```python
from build123d import *


with BuildPart() as part:
    # Sketch1 → Revolve1 (revolve)
    with BuildSketch(Plane.XY, mode=Mode.PRIVATE) as revolve1_sk:
        with BuildLine():
            Line((-4.9, 0), (-4.80754717, 3.5))
            Line((-4.80754717, 3.5), (-4.6, 3.5))
            Line((-4.6, 3.5), (-4.6, 4))
            Line((-4.6, 4), (-4.794339623, 4))
            Line((-4.794339623, 4), (-4.203177883, 26.379694424))
            ThreePointArc((-4.203177883, 26.379694424), (-4.171478034, 26.482572984), (-4.09103814, 26.554115293))
            ThreePointArc((-4.09103814, 26.554115293), (-2.09948154, 27.260450279), (0, 27.5))
            Line((0, 27.5), (0, 26.379694424))
            Line((0, 26.379694424), (-3.25, 26.379694424))
            Line((-3.25, 26.379694424), (-3.75, 1))
            Line((-3.75, 1), (-4, 1))
            Line((-4, 1), (-4, 0))
            Line((-4, 0), (-4.9, 0))
        make_face()
    revolve(revolve1_sk.sketch.rotate(Axis((0, 0, 0), (0, 1, 0)), 270), axis=Axis((0, 0, 0), (0, 1, 0)))


solid = part.part
```
Here's how the part is built. I have some questions about the finished solid (model axes, mm). A direction names the side the tool comes from. Round coordinates to 2 decimals unless told otherwise and drop trailing zeros. Loops run counter-clockwise (first coordinate to the right, second up) from the corner with the lowest first, then second, coordinate; pieces in that order, holes last. Notation, with made-up numbers: (4, 16) -> (22, 16) arc R19 cw to (22, 22) -> close; hole circle Ø5 at (43, 39.25). An arc over 180 degrees is marked (long way). Answer as CSV lines item,"result".
1. If we section it at B-B on y = 2.5: Please give me the cut outline in (x, z).
Final values:
outline,"circle Ø9.67 at (0, 0); hole circle Ø7.44 at (0, 0)"
2. Which directions (+Z, -Z, +X, -X, +Y, -Y) give clear straight access to the entire face, cutting with the end or side of a thin tool? Please do faces 1 (the face through (3.905, 0.493, 0.867)), 2 (the face through (4.74, 1.77, 1.05)).
Final values:
face 1,"-Y"
face 2,"+Y"
3. Thinking about a two-plate mould opening in Z: for faces 3 (the face through (-1.38, 3.75, -4.39)), 4 (the face through (4, 0, -2)), 5 (the face through (2.13, 13.51, 2.78)), 6 (the face through (0, 26.38, 0)), which applies, released by +Z, released by -Z, zero draft, split by the parting line, or undercut?
Final values:
face 3,"split by the parting line"
face 4,"zero draft"
face 5,"undercut"
face 6,"undercut"
4. If we section it at A-A on y = 14: Please give me the cut outline in (x, z), plus the area to 3 significant figures.
Final values:
outline,"circle Ø9.06 at (0, 0); hole circle Ø6.99 at (0, 0)"
area,"26.1 mm^2"
5. If I drill on L1, parallel to Z at x = 2, y = 6.75; L2, parallel to Z at x = 2.25, y = 7.75; L3, parallel to X at y = 0.3, z = 0, over which ranges is the centre line in solid material (lowest first)?
Final values:
L1,"z = -4.28 to -3.04, 3.04 to 4.28"
L2,"z = -4.12 to -2.83, 2.83 to 4.12"
L3,"x = -4.89 to -4, 4 to 4.89"
6. For pin 1 (5 mm diameter, centred on x = -1, y = 5.5, fed in from -Z); pin 2 (2 mm diameter, centred on x = -2, z = -1, fed in from +Y); pin 3 (5 mm diameter, centred on x = 0, z = 0, fed in from -Y), each with a flat end and sliding along its axis, tell me the tip position at first contact or that it passes through.
Final values:
pin 1,"stops at z = -4.82"
pin 2,"stops at y = 27.42"
pin 3,"stops at y = 26.38"
